Source: CAD feature listing. Evaluate the final solid. Frame: model axes, mm. A direction names the side the tool comes from. Give positions to 0.01 mm unless a question says otherwise; leave off trailing zeros. Answer in a Markdown table with one row per item.
```python
from build123d import *

# Parameters (mm, degrees)
SKETCH1_R           = 60
BOSS_EXTRUDE1_DEPTH = 10
SKETCH2_R           = 55
BOSS_EXTRUDE2_DEPTH = 7
SKETCH3_R           = 42.5
CUT_EXTRUDE1_DEPTH  = 87.539008545
SKETCH4_R           = 55
CUT_EXTRUDE2_DEPTH  = 3
SKETCH5_R           = 50
CUT_EXTRUDE3_DEPTH  = 11
SKETCH6_OUTSIDE_W   = 156.11
SKETCH6_OUTSIDE_H   = 156.11
SKETCH6_OUTSIDE_R   = 58.25
CUT_EXTRUDE4_DEPTH  = 3.2
CHAMFER1_SIZE       = 0.5
CHAMFER2_SIZE       = 0.5


with BuildPart() as part:
    # Sketch1 → Boss-Extrude1 (new body)
    with BuildSketch(Plane(origin=(0, 0, 0), x_dir=(1, 0, 0), z_dir=(0, 1, 0))):
        with Locations(Location((0, 0, 0), (0, 0, 270))):
            Circle(SKETCH1_R)
    extrude(amount=BOSS_EXTRUDE1_DEPTH)

    # Sketch2 → Boss-Extrude2 (add)
    with BuildSketch(Plane(origin=(0, 10, 0), x_dir=(1, 0, 0), z_dir=(0, 1, 0))):
        with Locations(Location((0, 0, 0), (0, 0, 270))):
            Circle(SKETCH2_R)
    extrude(amount=BOSS_EXTRUDE2_DEPTH)

    # Sketch3 → Cut-Extrude1 (cut, through all)
    with BuildSketch(Plane(origin=(0, 17, 0), x_dir=(1, 0, 0), z_dir=(0, 1, 0))):
        with Locations(Location((0, 0, 0), (0, 0, 270))):
            Circle(SKETCH3_R)
    extrude(amount=-CUT_EXTRUDE1_DEPTH, mode=Mode.SUBTRACT)

    # Sketch4 → Cut-Extrude2 (cut)
    with BuildSketch(Plane.XZ):
        with Locations(Location((0, 0, 0), (0, 0, 90))):
            Circle(SKETCH4_R)
    extrude(amount=-CUT_EXTRUDE2_DEPTH, mode=Mode.SUBTRACT)

    # Sketch5 → Cut-Extrude3 (cut)
    with BuildSketch(Plane.XZ.offset(-3)):
        with Locations(Location((0, 0, 0), (0, 0, 270))):
            Circle(SKETCH5_R)
    extrude(amount=-CUT_EXTRUDE3_DEPTH, mode=Mode.SUBTRACT)

    # Sketch6 outside → Cut-Extrude4 (cut)
    with BuildSketch(Plane(origin=(0, 6, 0), x_dir=(-1, 0, 0), z_dir=(0, -1, 0))):
        Rectangle(SKETCH6_OUTSIDE_W, SKETCH6_OUTSIDE_H)
        with Locations(Location((0, 0, 0), (0, 0, 90))):
            Circle(SKETCH6_OUTSIDE_R, mode=Mode.SUBTRACT)
    extrude(amount=CUT_EXTRUDE4_DEPTH, mode=Mode.SUBTRACT)

    # Chamfer1
    chamfer1_edges = [part.edges().sort_by_distance(p)[0] for p in [
        (0, 0, -60),
    ]]
    chamfer(chamfer1_edges, length=CHAMFER1_SIZE)

    # Chamfer2
    chamfer2_edges = [part.edges().sort_by_distance(p)[0] for p in [
        (0, 17, -55),
    ]]
    chamfer(chamfer2_edges, length=CHAMFER2_SIZE)


solid = part.part
```
(1) Access query for faces 1 (the cylindrical face through (-48.794, 13.204, 25.379)), 2 (the flat face through (9, 2.8, -58)), 3 (the cylindrical face through (-25.861, 15.521, -33.727)), 4 (the flat face through (49, 3, 12)). Directions: +Z, -Z, +X, -X, +Y, -Y. A direction counts if a zero-diameter tool reaches every point of the face in a straight line with its end or side. Return the directions, or none.
A:
| item | result |
|---|---|
| face 1 | +Y |
| face 2 | none |
| face 3 | +Y, -Y |
| face 4 | -Y |
(2) First-contact query: pin 1 Ø10 at (x, y) = (-4.5, 10.5) entering from -Z; pin 2 Ø4 at (y, z) = (9.5, 11) entering from -X; pin 3 Ø5 at (x, y) = (-7.5, 8.5) entering from +Z; pin 4 Ø10 at (x, y) = (14, 3) entering from -Z. Flat tips, straight axial feed; report the tip coordinate or a pass-through.
A:
| item | result |
|---|---|
| pin 1 | stops at z = -60 |
| pin 2 | stops at x = -59.32 |
| pin 3 | stops at z = 59.79 |
| pin 4 | stops at z = -59.32 |
(3) Ray query, probe 1 along Y at (x, z) = (-49.5, 31); probe 2 along X at (y, z) = (7.75, -0.5); probe 3 along X at (y, z) = (14.7, 0). Return the intervals inside material, ascending.
A:
| item | result |
|---|---|
| probe 1 | y = 0 to 2.8, 6 to 10 |
| probe 2 | x = -60 to -50, 50 to 60 |
| probe 3 | x = -55 to -42.5, 42.5 to 55 |
(4) Pull-direction query (Y, two-part tool) for faces 5 (the flat face through (-53, 0, 17)), 6 (the flat face through (9, 6, -58)), 7 (the flat face through (-32, 17, -29)), 8 (the cylindrical face through (48.794, 1.479, 25.379)); classes: +Y half, -Y half, draft (parallel to the pull), parting line (faces both ways), or undercut.
A:
| item | result |
|---|---|
| face 5 | -Y half |
| face 6 | undercut |
| face 7 | +Y half |
| face 8 | draft |
